from build123d import *

# Parameters (mm, degrees)
EXTRUDE_3_DEPTH     = 5
SKETCH_2_W          = 12
SKETCH_2_H          = 20
EXTRUDE_4_DEPTH     = 50
CUT_EXTRUDE_1_DEPTH = 5
SKETCH_4_W          = 112
SKETCH_4_H          = 5
EXTRUDE_5_DEPTH     = 40
CUT_EXTRUDE_2_REACH = 1236.326
SKETCH_5_R          = 6
SKETCH_5_R_2        = 5
CUT_EXTRUDE_3_REACH = 1236.529
SKETCH_6_R          = 7.332886018
SKETCH_6_R_2        = 7.301331484
SKETCH_6_R_3        = 6.603217824


with BuildPart() as part:
    # 草图1 → 凸台-拉伸3 (new body)
    with BuildSketch(Plane.XY):
        with BuildLine():
            Line((-86.707495778, -188.910549606), (103.292504222, -188.910549606))
            Line((103.292504222, -188.910549606), (103.292504222, 44.089450394))
            ThreePointArc((103.292504222, 44.089450394), (71.593223998, 37.797700493), (44.699821924, 19.876333124))
            add(Edge.make_bspline(
                [(-10.94366291, -38.46742639), (16.878079507, -9.295546633), (44.699821924, 19.876333124)],
                knots=[-0.0017101, -0.0017101, -0.0017101, 0.998178008, 0.998178008, 0.998178008], degree=2))
            ThreePointArc((-10.94366291, -38.46742639), (-45.692777784, -61.737635508), (-86.707495778, -69.910549606))
            Line((-86.707495778, -69.910549606), (-166.707495778, -69.910549606))
            Line((-166.707495778, -69.910549606), (-166.707495778, -188.910549606))
            Line((-166.707495778, -188.910549606), (-86.707495778, -188.910549606))
        make_face()
    extrude(amount=EXTRUDE_3_DEPTH)

    # 草图2 → 凸台-拉伸4 (add)
    with BuildSketch(Plane(origin=(0, -69.910549606, 0), x_dir=(1, 0, 0), z_dir=(0, 1, 0))):
        with Locations((-172.707495778, 5)):
            Rectangle(SKETCH_2_W, SKETCH_2_H)
    extrude(amount=-EXTRUDE_4_DEPTH)

    # 草图3 → 切除-拉伸1 (cut)
    with BuildSketch(Plane(origin=(0, -69.910549606, 0), x_dir=(1, 0, 0), z_dir=(0, 1, 0))):
        Polygon((-166.707495778, 0), (-166.707495778, -5), (-176.720177385, -5), (-176.720177385, 7.5), (-178.707495778, 7.5), (-178.707495778, 15), (-166.707495778, 15), align=None)
    extrude(amount=-CUT_EXTRUDE_1_DEPTH, mode=Mode.SUBTRACT)

    # 草图4 → 凸台-拉伸5 (add)
    with BuildSketch(Plane.XZ.offset(188.910549606)):
        with Locations((47.292504222, 2.5)):
            Rectangle(SKETCH_4_W, SKETCH_4_H)
    extrude(amount=EXTRUDE_5_DEPTH)

    # 草图5 → 切除-拉伸2 (cut, up to next)
    with BuildSketch(Plane(origin=(703.41878585, 634.231928171, 5), x_dir=(0, 1, 0), z_dir=(0, 0, 1)), mode=Mode.PRIVATE) as cut_extrude_2_sk1:
        with Locations(Location((-666.704267343, 635.126281628, 0), (0, 0, 270))):
            Circle(SKETCH_5_R)
    cut_extrude_2_tool1 = extrude(cut_extrude_2_sk1.sketch, amount=-CUT_EXTRUDE_2_REACH, mode=Mode.PRIVATE) & part.part
    # 草图5 → 切除-拉伸2 (cut, up to next)
    with BuildSketch(Plane(origin=(703.41878585, 634.231928171, 5), x_dir=(0, 1, 0), z_dir=(0, 0, 1)), mode=Mode.PRIVATE) as cut_extrude_2_sk2:
        with Locations(Location((-746.704267343, 635.126281628, 0), (0, 0, 270))):
            Circle(SKETCH_5_R_2)
    cut_extrude_2_tool2 = extrude(cut_extrude_2_sk2.sketch, amount=-CUT_EXTRUDE_2_REACH, mode=Mode.PRIVATE) & part.part
    # 草图5 → 切除-拉伸2 (cut, up to next)
    with BuildSketch(Plane(origin=(703.41878585, 634.231928171, 5), x_dir=(0, 1, 0), z_dir=(0, 0, 1)), mode=Mode.PRIVATE) as cut_extrude_2_sk3:
        with Locations(Location((-746.704267343, 840.126281628, 0), (0, 0, 270))):
            Circle(SKETCH_5_R)
    cut_extrude_2_tool3 = extrude(cut_extrude_2_sk3.sketch, amount=-CUT_EXTRUDE_2_REACH, mode=Mode.PRIVATE) & part.part
    # 草图5 → 切除-拉伸2 (cut, up to next)
    with BuildSketch(Plane(origin=(703.41878585, 634.231928171, 5), x_dir=(0, 1, 0), z_dir=(0, 0, 1)), mode=Mode.PRIVATE) as cut_extrude_2_sk4:
        with Locations(Location((-746.704267343, 735.126281628, 0), (0, 0, 270))):
            Circle(SKETCH_5_R)
    cut_extrude_2_tool4 = extrude(cut_extrude_2_sk4.sketch, amount=-CUT_EXTRUDE_2_REACH, mode=Mode.PRIVATE) & part.part
    add(cut_extrude_2_tool1.solids().sort_by_distance((68.292504, -32.472339, 5))[0], mode=Mode.SUBTRACT)
    add(cut_extrude_2_tool2.solids().sort_by_distance((68.292504, -112.472339, 5))[0], mode=Mode.SUBTRACT)
    add(cut_extrude_2_tool3.solids().sort_by_distance((-136.707496, -112.472339, 5))[0], mode=Mode.SUBTRACT)
    add(cut_extrude_2_tool4.solids().sort_by_distance((-31.707496, -112.472339, 5))[0], mode=Mode.SUBTRACT)

    # 草图6 → 切除-拉伸3 (cut, up to next)
    with BuildSketch(Plane(origin=(703.41878585, 634.231928171, 15), x_dir=(0, 1, 0), z_dir=(0, 0, 1)), mode=Mode.PRIVATE) as cut_extrude_3_sk1:
        with Locations(Location((-804.642477777, 640.126281628, 0), (0, 0, 270))):
            Circle(SKETCH_6_R)
    cut_extrude_3_tool1 = extrude(cut_extrude_3_sk1.sketch, amount=-CUT_EXTRUDE_3_REACH, mode=Mode.PRIVATE) & part.part
    # 草图6 → 切除-拉伸3 (cut, up to next)
    with BuildSketch(Plane(origin=(703.41878585, 634.231928171, 15), x_dir=(0, 1, 0), z_dir=(0, 0, 1)), mode=Mode.PRIVATE) as cut_extrude_3_sk2:
        with Locations(Location((-804.642477777, 710.126281628, 0), (0, 0, 270))):
            Circle(SKETCH_6_R_2)
    cut_extrude_3_tool2 = extrude(cut_extrude_3_sk2.sketch, amount=-CUT_EXTRUDE_3_REACH, mode=Mode.PRIVATE) & part.part
    # 草图6 → 切除-拉伸3 (cut, up to next)
    with BuildSketch(Plane(origin=(703.41878585, 634.231928171, 15), x_dir=(0, 1, 0), z_dir=(0, 0, 1)), mode=Mode.PRIVATE) as cut_extrude_3_sk3:
        with Locations(Location((-804.642477777, 780.126281628, 0), (0, 0, 270))):
            Circle(SKETCH_6_R_3)
    cut_extrude_3_tool3 = extrude(cut_extrude_3_sk3.sketch, amount=-CUT_EXTRUDE_3_REACH, mode=Mode.PRIVATE) & part.part
    add(cut_extrude_3_tool1.solids().sort_by_distance((63.292504, -170.41055, 15))[0], mode=Mode.SUBTRACT)
    add(cut_extrude_3_tool2.solids().sort_by_distance((-6.707496, -170.41055, 15))[0], mode=Mode.SUBTRACT)
    add(cut_extrude_3_tool3.solids().sort_by_distance((-76.707496, -170.41055, 15))[0], mode=Mode.SUBTRACT)


solid = part.part
Source: CAD feature listing. Evaluate the final solid. Frame: model axes, mm. A direction names the side the tool comes from. Coordinates: 2 decimals unless noted, no trailing zeros. Order: outer loops, then holes, each group sorted by start corner. A loop starts at its lowest first (then second) coordinate and runs counter-clockwise, first axis right, second up.
Item 1: Cut plane B-B (z = -4.25). Return loops of the section in (x, y), plus the area to 3 significant figures.
Output values:
outline: (-178.71, -119.91) - (-166.71, -119.91) - (-166.71, -74.91) - (-176.72, -74.91) - (-176.72, -69.91) - (-178.71, -69.91) - close
area: 550 mm2
Item 2: Cut plane A-A (x = -76.5). Return loops of the section in (y, z), plus the area to 3 significant figures.
Output values:
outline: (-188.91, 0) - (-177.01, 0) - (-177.01, 5) - (-188.91, 5) - close; (-163.81, 0) - (-69.42, 0) - (-69.42, 5) - (-163.81, 5) - close
area: 531 mm2
Item 3: Pull-direction query (Y, two-part tool) for faces 3 (the face through (-178.707, -95, -5)), 4 (the face through (72.01, 37.97, 2.46)), 5 (the face through (-173, -119.911, -5)), 6 (the face through (73.835, -34.77, 2.535)); classes: pulls with the +Y half, pulls with the -Y half, needs draft (parallel to the pull), parting line crosses it, or undercut.
Output values:
face 3: needs draft
face 4: pulls with the +Y half
face 5: pulls with the -Y half
face 6: undercut
Item 4: Cut plane C-C (y = -80.5). Return loops of the section in (x, z), plus the area to 3 significant figures.
Output values:
outline: (-178.71, -15) - (-166.71, -15) - (-166.71, 0) - (103.29, 0) - (103.29, 5) - (-178.71, 5) - close
area: 1,590 mm2
Item 5: Set-up query: faces 1 (the face through (-166.707, -97, -7)), 2 (the face through (-141.13, -108.42, 2.54)). Return all of +Z, -Z, +X, -X, +Y, -Y with unobstructed straight access to the full face (end or side cutting, diameter ignored); none if empty.
Output values:
face 1: -Z, +X, +Y, -Y
face 2: +Z, -Z
Item 6: Cut plane D-D (x = -112). Return loops of the section in (y, z), plus the area to 3 significant figures.
Output values:
outline: (-188.91, 0) - (-69.91, 0) - (-69.91, 5) - (-188.91, 5) - close
area: 595 mm2
Item 7: First-contact query: P1, Ø5.5, axis at y = -165, z = 1.5, coming from the -X side; P2, Ø1, axis at x = -177, y = -72, coming from the -Z side; P3, Ø12, axis at x = -127, y = -76.5, coming from the -Z side; P4, Ø15, axis at x = -76.71, y = -170.41, coming from the +Z side. Flat tips, straight axial feed; report the tip coordinate or a pass-through.
Output values:
P1: stops at x = -166.71
P2: stops at z = -7.5
P3: stops at z = 0
P4: stops at z = 5
Item 8: Material intervals for line 1 (Z direction, x = -107.5, y = -71.5); line 2 (Y direction, x = -157.5, z = 4.25); line 3 (Y direction, x = -27, z = 0.75), sorted ascending.
Output values:
line 1: z = 0 to 5
line 2: y = -188.91 to -69.91
line 3: y = -188.91 to -116.19, -108.75 to -51.7
